The drawing under review shows one solid part. Ordinate dimensions are in mm from its lowest x, y, z. Coordinates: 2 decimals unless noted, no trailing zeros. Write each loop counter-clockwise with the first axis right and the second up, starting at its lowest first coordinate (ties: lowest second). Pieces come first, ordered by that corner, then holes. Notation, with made-up numbers: (25, 48.5) - (60, 48.5) arc R28 ccw to (60, 84.5) - close; hole circle Ø4 at (39, -39.5). An arc over 180 degrees is marked (long way). Answer as CSV lines item,"result". Start each with the question number.
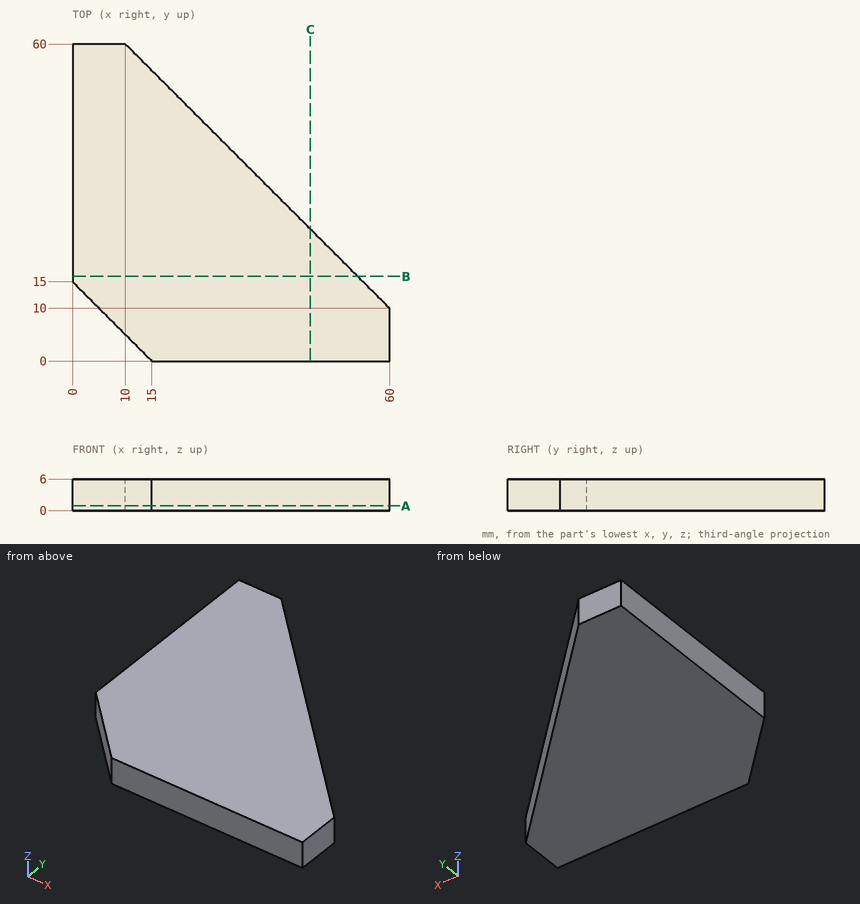
(1) For pin 1 (4 mm diameter, centred on x = 24, y = 34.5, fed in from -Z); pin 2 (1 mm diameter, centred on x = 32, z = 1.5, fed in from +Y), all flat-tipped, find the tip position at first contact; note any pin that passes through.
(2) Add section A-A on z = 0.9. Give the boundary of the cut face in (x, y), then the cut area to 3 significant figures.
(3) Wall thickness on line 1 (Y direction, x = 55, z = 3.65); line 2 (Y direction, x = 5, z = 2.75); line 3 (X direction, y = 22.5, z = 2.85): over which ranges is each line inside the solid? List them lowest first.
(4) Add section C-C on x = 45. Give the boundary of the cut face in (y, z), then the cut area to 3 significant figures.
(5) Add section B-B on y = 16. Give the boundary of the cut face in (x, z).
Reported:
1,pin 1,"z = 0"
1,pin 2,"y = 38.5"
2,outline,"(0, 15) - (15, 0) - (60, 0) - (60, 10) - (10, 60) - (0, 60) - close"
2,area,"2,240 mm²"
3,line 1,"0 to 15"
3,line 2,"10 to 60"
3,line 3,"0 to 47.5"
4,outline,"(0, 0) - (25, 0) - (25, 6) - (0, 6) - close"
4,area,"150 mm²"
5,outline,"(0, 0) - (54, 0) - (54, 6) - (0, 6) - close"
